Model file for the job. Use its own axes, mm. Round coordinates to 2 decimals unless told otherwise and drop trailing zeros. Order: outer loops, then holes, each group sorted by start corner. A loop starts at its lowest first (then second) coordinate and runs counter-clockwise, first axis right, second up. Notation, with made-up numbers: (-10, -35) - (22, -35) arc R31 cw to (22, -3) - close; hole circle Ø10 at (50, 37.25). An arc over 180 degrees is marked (long way). Put each result on its own line as item: value. Start each with the question number.
Item 1: Probe probe 1 along X at (y, z) = (-19, -717.5); probe 2 along Y at (x, z) = (23.1, -270). List the from-to ranges inside material, lowest first.
Item 2: Saw through at A-A on z = -869. List the corners of the cut face in (x, y).
Item 3: Saw through at B-B on x = 0. List the corners of the cut face in (y, z), plus the area to 3 significant figures.
Item 4: Pin check, flat tip, straight feed: pin 1 Ø3 at (y, z) = (15, -15) entering from +X. Stop position of the tip, or through.
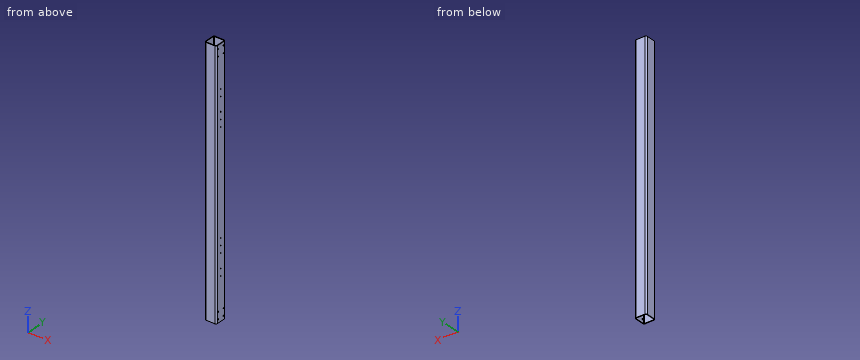
```python
from build123d import *

# Parameters (mm, degrees)
GB_6728_1986_050_X_50_X_3_1_DEPTH = 1100
HOLE_WIZARD_M5_1_D                = 4.2
HOLE_WIZARD_M5_1_DEPTH            = 12.4
HOLE_WIZARD_M5_1_TIP              = 1.2618073
HOLE_WIZARD_M5_2_D                = 4.2
HOLE_WIZARD_M5_2_DEPTH            = 15
HOLE_WIZARD_M5_2_TIP              = 1.2618073
HOLE_WIZARD_M5_3_D                = 4.2
HOLE_WIZARD_M5_3_DEPTH            = 12.4
HOLE_WIZARD_M5_3_TIP              = 1.2618073
HOLE_WIZARD_M6_1_D                = 5
HOLE_WIZARD_M6_1_DEPTH            = 15
HOLE_WIZARD_M6_1_TIP              = 1.502151548


with BuildPart() as part:
    # Sketch1 → Gb／6728-1986方形空心型钢 050 X 50 X 3(1) (new body)
    with BuildSketch(Plane(origin=(0, 0, 0), x_dir=(-1, 0, 0), z_dir=(0, 0, -1))):
        with BuildLine():
            Line((-19, -25), (19, -25))
            ThreePointArc((19, -25), (23.242640687, -23.242640687), (25, -19))
            Line((25, -19), (25, 19))
            ThreePointArc((25, 19), (23.242640687, 23.242640687), (19, 25))
            Line((19, 25), (-19, 25))
            ThreePointArc((-19, 25), (-23.242640687, 23.242640687), (-25, 19))
            Line((-25, 19), (-25, -19))
            ThreePointArc((-25, -19), (-23.242640687, -23.242640687), (-19, -25))
        make_face()
        with BuildLine():
            Line((-19, -22), (19, -22))
            ThreePointArc((19, -22), (21.121320344, -21.121320344), (22, -19))
            Line((22, -19), (22, 19))
            ThreePointArc((22, 19), (21.121320344, 21.121320344), (19, 22))
            Line((19, 22), (-19, 22))
            ThreePointArc((-19, 22), (-21.121320344, 21.121320344), (-22, 19))
            Line((-22, 19), (-22, -19))
            ThreePointArc((-22, -19), (-21.121320344, -21.121320344), (-19, -22))
        make_face(mode=Mode.SUBTRACT)
    extrude(amount=GB_6728_1986_050_X_50_X_3_1_DEPTH)

    # M5 螺纹孔1
    with Locations(Plane(origin=(25, 0, 0), x_dir=(0, 0, -1), z_dir=(1, 0, 0))):
        with Locations((180, 0), (210, 0)):
            Hole(HOLE_WIZARD_M5_1_D / 2, depth=HOLE_WIZARD_M5_1_DEPTH)
            with Locations((0, 0, -(HOLE_WIZARD_M5_1_DEPTH + HOLE_WIZARD_M5_1_TIP / 2))):  # 118° drill point
                Cone(0, HOLE_WIZARD_M5_1_D / 2, HOLE_WIZARD_M5_1_TIP, mode=Mode.SUBTRACT)

    # M5 螺纹孔2
    with Locations(Plane(origin=(25, 0, 0), x_dir=(0, 0, -1), z_dir=(1, 0, 0))):
        with Locations((270, 0), (300, 0), (330, 0)):
            Hole(HOLE_WIZARD_M5_2_D / 2, depth=HOLE_WIZARD_M5_2_DEPTH)
            with Locations((0, 0, -(HOLE_WIZARD_M5_2_DEPTH + HOLE_WIZARD_M5_2_TIP / 2))):  # 118° drill point
                Cone(0, HOLE_WIZARD_M5_2_D / 2, HOLE_WIZARD_M5_2_TIP, mode=Mode.SUBTRACT)

    # M5 螺纹孔3
    with Locations(Plane(origin=(25, 0, 0), x_dir=(0, 0, -1), z_dir=(1, 0, 0))):
        with Locations((920, 0), (890, 0), (830, 0), (800, 0), (770, 0)):
            Hole(HOLE_WIZARD_M5_3_D / 2, depth=HOLE_WIZARD_M5_3_DEPTH)
            with Locations((0, 0, -(HOLE_WIZARD_M5_3_DEPTH + HOLE_WIZARD_M5_3_TIP / 2))):  # 118° drill point
                Cone(0, HOLE_WIZARD_M5_3_D / 2, HOLE_WIZARD_M5_3_TIP, mode=Mode.SUBTRACT)

    # M6 螺纹孔1
    with Locations(Plane(origin=(25, 0, 0), x_dir=(0, 0, -1), z_dir=(1, 0, 0))):
        with Locations((15, 15), (45, 15), (15, -15), (45, -15), (1055, 15), (1085, 15), (1055, -15), (1085, -15)):
            Hole(HOLE_WIZARD_M6_1_D / 2, depth=HOLE_WIZARD_M6_1_DEPTH)
            with Locations((0, 0, -(HOLE_WIZARD_M6_1_DEPTH + HOLE_WIZARD_M6_1_TIP / 2))):  # 118° drill point
                Cone(0, HOLE_WIZARD_M6_1_D / 2, HOLE_WIZARD_M6_1_TIP, mode=Mode.SUBTRACT)


solid = part.part
```
Results found:
1. probe 1: x = -25 to -22, 22 to 25
1. probe 2: y = -23.38 to -2.1, 2.1 to 23.38
2. outline: (-25, -19) arc R6 ccw to (-19, -25) - (19, -25) arc R6 ccw to (25, -19) - (25, 19) arc R6 ccw to (19, 25) - (-19, 25) arc R6 ccw to (-25, 19) - close; hole (-22, -19) arc R3 ccw to (-19, -22) - (19, -22) arc R3 ccw to (22, -19) - (22, 19) arc R3 ccw to (19, 22) - (-19, 22) arc R3 ccw to (-22, 19) - close
3. outline: (-25, -1100) - (-22, -1100) - (-22, 0) - (-25, 0) - close; (22, -1100) - (25, -1100) - (25, 0) - (22, 0) - close
3. area: 6,600 mm²
4. pin 1: stops at x = -22
